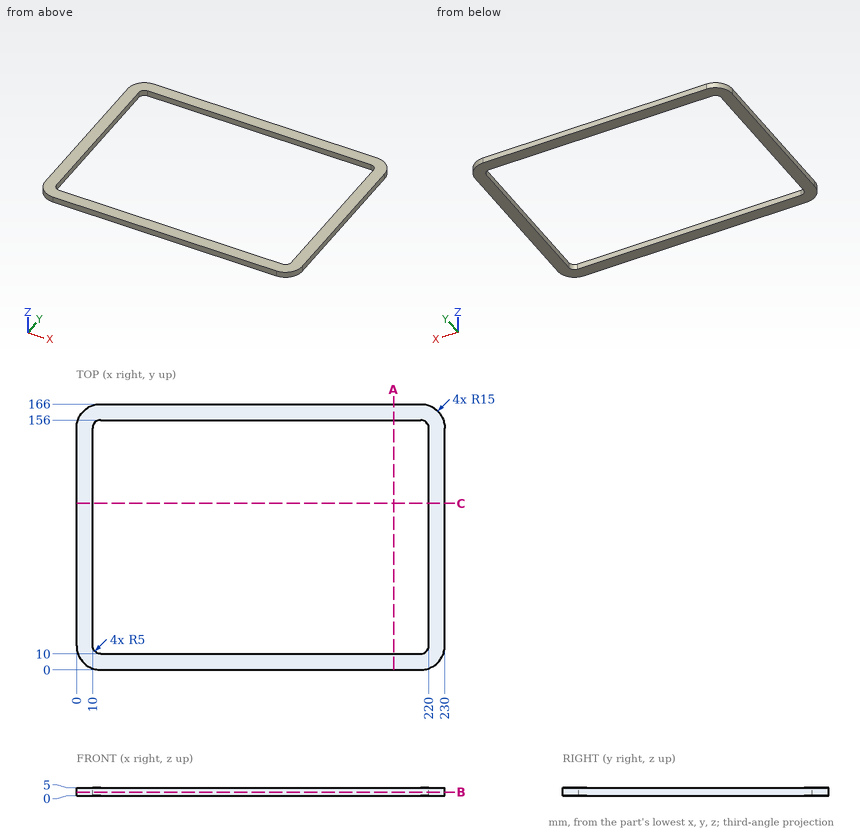
Study the drawing (mm; zero at the part's minimum x, y, z) and answer. Give positions to 0.01 mm unless a question says otherwise; leave off trailing zeros. Order: outer loops, then holes, each group sorted by start corner. A loop starts at its lowest first (then second) coordinate and runs counter-clockwise, first axis right, second up.
1) Given P1, Ø12, axis at x = 166.5, y = 145, coming from the +Z side; P2, Ø2.5, axis at y = 71, z = 3.5, coming from the -X side, each flat-ended and moving along its own axis, determine where each tip first touches the part or whether it passes through.
Reported:
P1: passes through
P2: stops at x = 0
2) Find section A-A on x = 198. Write down the section's boundary in (y, z), then the cut area to 3 significant figures.
Reported:
outline: (0, 0) - (10, 0) - (10, 5) - (0, 5) - close; (156, 0) - (166, 0) - (166, 5) - (156, 5) - close
area: 100 mm2
3) Consider line 1 along X through (y, z) = (57, 2.6); line 2 along Y through (x, z) = (125.5, 0.9); line 3 along Y through (x, z) = (9.5, 4.1). Determine where each line is inside the solid, lowest interval first.
Reported:
line 1: x = 0 to 10, 220 to 230
line 2: y = 0 to 10, 156 to 166
line 3: y = 1.04 to 164.96
4) Find section C-C on y = 104. Write down the section's boundary in (x, z), then the cut area to 3 significant figures.
Reported:
outline: (0, 0) - (10, 0) - (10, 5) - (0, 5) - close; (220, 0) - (230, 0) - (230, 5) - (220, 5) - close
area: 100 mm2
5) Find section B-B on z = 2.25. Write down the section's boundary in (x, y), then the cut area to 3 significant figures.
Reported:
outline: (0, 15) arc R15 ccw to (15, 0) - (215, 0) arc R15 ccw to (230, 15) - (230, 151) arc R15 ccw to (215, 166) - (15, 166) arc R15 ccw to (0, 151) - close; hole (10, 15) arc R5 ccw to (15, 10) - (215, 10) arc R5 ccw to (220, 15) - (220, 151) arc R5 ccw to (215, 156) - (15, 156) arc R5 ccw to (10, 151) - close
area: 7,350 mm2
